Verification items for the finished model (mm, model axes). A direction names the side the tool comes from. Round coordinates to 2 decimals unless told otherwise and drop trailing zeros. Write each loop counter-clockwise with the first axis right and the second up, starting at its lowest first coordinate (ties: lowest second). Pieces come first, ordered by that corner, then holes. Notation, with made-up numbers: M 29,-32.5 L 45,-32.5 A17 cw 45,0.5 Z; hole C 82,69 d5. An arc over 180 degrees is marked long. One line per question, with ' | ' between items.
from build123d import *

# Parameters (mm, degrees)
SKETCH1_R           = 51.5
SKETCH1_R_2         = 41.5
BOSS_EXTRUDE1_DEPTH = 8
CIRPATTERN1_COUNT   = 4


with BuildPart() as part:
    # Sketch1 → Boss-Extrude1 (new body)
    with BuildSketch(Plane.XY):
        Circle(SKETCH1_R)
        Circle(SKETCH1_R_2, mode=Mode.SUBTRACT)
    extrude(amount=BOSS_EXTRUDE1_DEPTH)

    # Sketch5 → Hole size per hex socket cap screw type1 (revolve, cut)
    with BuildSketch(Plane(origin=(0, 46.5, 8), x_dir=(0, -1, 0), z_dir=(1, 0, 0))):
        Polygon((0, 0), (0, 18.351936393), (2.25, 17), (2.25, 4.6), (4, 4.6), (4, 0), align=None)
    hole_size_per_hex_socket_cap_screw_type1 = revolve(axis=Axis((0, 46.5, 14.35), (0, 0, -1)), mode=Mode.SUBTRACT)

    # CirPattern1: Hole size per hex socket cap screw type1 ×4 about axis
    cirpattern1_axis = Axis((0, 0, 0), (0, 0, 1))
    for i in range(1, CIRPATTERN1_COUNT):
        add(hole_size_per_hex_socket_cap_screw_type1.rotate(cirpattern1_axis, i * 360 / CIRPATTERN1_COUNT), mode=Mode.SUBTRACT)


solid = part.part
1. Section check A-A, the plane x = 0. Record the cut outline in (y, z), then the cut area to 3 significant figures.
Results:
outline: M -51.5,0 L -48.75,0 L -48.75,3.4 L -50.5,3.4 L -50.5,8 L -51.5,8 Z; M -44.25,0 L -41.5,0 L -41.5,8 L -42.5,8 L -42.5,3.4 L -44.25,3.4 Z; M 41.5,0 L 44.25,0 L 44.25,3.4 L 42.5,3.4 L 42.5,8 L 41.5,8 Z; M 48.75,0 L 51.5,0 L 51.5,8 L 50.5,8 L 50.5,3.4 L 48.75,3.4 Z | area: 55.8 mm2
2. Tool access check on faces 1 (the face through (-0.099, 48.748, 1.724)), 2 (the face through (-2, -48, 3.4)). Record the directions out of +Z, -Z, +X, -X, +Y, -Y that give a thin tool (end or side, any length) a straight path to the whole face; none if there is none.
Results:
face 1: +Z, -Z | face 2: +Z
3. Section check C-C, the plane z = 5. Record the cut outline in (x, y).
Results:
outline: C 0,0 d103; hole C -46.5,0 d8; hole C 0,0 d83; hole C 0,-46.5 d8; hole C 0,46.5 d8; hole C 46.5,0 d8
4. Mould release check, pull along Y, two halves, no side actions. Record for faces 3 (the face through (4, -42, 8)), 4 (the face through (48, -2, 3.4)), 5 (the face through (-11.164, -50.275, 3.944)): pulls with the +Y half, pulls with the -Y half, needs draft (parallel to the pull), parting line crosses it, or undercut.
Results:
face 3: needs draft | face 4: undercut | face 5: parting line crosses it
5. Section check D-D, the plane x = -35.5. Record the cut outline in (y, z), then the cut area to 3 significant figures.
Results:
outline: M -37.31,0 L -21.49,0 L -21.49,8 L -37.31,8 Z; M 21.49,0 L 37.31,0 L 37.31,8 L 21.49,8 Z | area: 253 mm2
6. Go/stop test with flat-tipped pins: P1, Ø3, axis at x = 40.5, z = 2, coming from the -Y side; P2, Ø3.5, axis at x = 0, y = -46.5, coming from the -Z side; P3, Ø1.5, axis at x = 35, z = 6, coming from the +Y side; P4, Ø2, axis at x = -22, z = 1, coming from the -Y side. Record where each tip stops, or that it passes through.
Results:
P1: stops at y = -33.63 | P2: passes through | P3: stops at y = 38.46 | P4: stops at y = -47.02
7. Thickness scan on line 1 (Y direction, x = 0, z = 2.25); line 2 (X direction, y = -17, z = 7.5); line 3 (Y direction, x = 4.5, z = 1.25). Record the ranges inside material, lowest first.
Results:
line 1: y = -51.5 to -48.75, -44.25 to -41.5, 41.5 to 44.25, 48.75 to 51.5 | line 2: x = -48.61 to -37.86, 37.86 to 48.61 | line 3: y = -51.3 to -41.26, 41.26 to 51.3
